from build123d import *

# Parameters (mm, degrees)
SKETCH_1_W                  = 30
SKETCH_1_H                  = 57
EXTRUDE_1_DEPTH             = 25
SKETCH_2_W                  = 5
SKETCH_2_H                  = 52
CUT_EXTRUDE_1_DEPTH         = 65.02343321
SKETCH_3_W                  = 5
SKETCH_3_H                  = 52
CUT_EXTRUDE_2_DEPTH         = 65.02343321
SKETCH_4_W                  = 20
SKETCH_4_H                  = 38
EXTRUDE_2_DEPTH             = 20
SKETCH_5_W                  = 28.836169251
SKETCH_5_H                  = 18
CUT_EXTRUDE_3_DEPTH         = 69.190018281
HOLE_WIZARD_10_0_10_1_D     = 10
HOLE_WIZARD_10_0_10_1_DEPTH = 10
HOLE_WIZARD_10_0_10_2_D     = 10
HOLE_WIZARD_10_0_10_2_DEPTH = 38
HOLE_WIZARD_5_0_5_1_D       = 5
HOLE_WIZARD_5_0_5_1_DEPTH   = 17
HOLE_WIZARD_5_0_5_1_TIP     = 1.502151548
CHAMFER_1_SIZE              = 1
CHAMFER_2_SIZE              = 10
FILLET_1_R                  = 5


with BuildPart() as part:
    # 草图1 → 凸台-拉伸1 (new body)
    with BuildSketch(Plane(origin=(17.145402657, 0, 0), x_dir=(0, 0, -1), z_dir=(1, 0, 0))):
        with Locations((0, 28.5)):
            Rectangle(SKETCH_1_W, SKETCH_1_H)
    extrude(amount=-EXTRUDE_1_DEPTH)

    # 草图2 → 切除-拉伸1 (cut, through all)
    with BuildSketch(Plane(origin=(17.145402657, 0, 0), x_dir=(0, 0, -1), z_dir=(1, 0, 0))):
        with Locations((-12.5, 31)):
            Rectangle(SKETCH_2_W, SKETCH_2_H)
    extrude(amount=-CUT_EXTRUDE_1_DEPTH, mode=Mode.SUBTRACT)

    # 草图3 → 切除-拉伸2 (cut, through all)
    with BuildSketch(Plane(origin=(17.145402657, 0, 0), x_dir=(0, 0, -1), z_dir=(1, 0, 0))):
        with Locations((12.5, 31)):
            Rectangle(SKETCH_3_W, SKETCH_3_H)
    extrude(amount=-CUT_EXTRUDE_2_DEPTH, mode=Mode.SUBTRACT)

    # 草图4 → 凸台-拉伸2 (add)
    with BuildSketch(Plane.ZY.offset(7.854597343)):
        with Locations((0, 38)):
            Rectangle(SKETCH_4_W, SKETCH_4_H)
    extrude(amount=EXTRUDE_2_DEPTH)

    # 草图5 → 切除-拉伸3 (cut, through all)
    with BuildSketch(Plane.XY.offset(10)):
        with Locations((-13.436512718, 38)):
            Rectangle(SKETCH_5_W, SKETCH_5_H)
    extrude(amount=-CUT_EXTRUDE_3_DEPTH, mode=Mode.SUBTRACT)

    # Ø10.0 (10) 直径孔1
    with Locations(Plane(origin=(0, 47, 0), x_dir=(-1, 0, 0), z_dir=(0, -1, 0))):
        with Locations((17.854597343, 0)):
            Hole(HOLE_WIZARD_10_0_10_1_D / 2, depth=HOLE_WIZARD_10_0_10_1_DEPTH)

    # Ø10.0 (10) 直径孔2
    with Locations(Plane(origin=(0, 19, 0), x_dir=(-1, 0, 0), z_dir=(0, -1, 0))):
        with Locations((17.854597343, 0)):
            Hole(HOLE_WIZARD_10_0_10_2_D / 2, depth=HOLE_WIZARD_10_0_10_2_DEPTH)

    # Ø5.0 (5) 直径孔1
    with Locations(Plane(origin=(0, 0, 0), x_dir=(-1, 0, 0), z_dir=(0, -1, 0))):
        with Locations((2.854597343, 0), (-12.145402657, 0)):
            Hole(HOLE_WIZARD_5_0_5_1_D / 2, depth=HOLE_WIZARD_5_0_5_1_DEPTH)
            with Locations((0, 0, -(HOLE_WIZARD_5_0_5_1_DEPTH + HOLE_WIZARD_5_0_5_1_TIP / 2))):  # 118° drill point
                Cone(0, HOLE_WIZARD_5_0_5_1_D / 2, HOLE_WIZARD_5_0_5_1_TIP, mode=Mode.SUBTRACT)

    # 倒角1
    chamfer_1_edges = [part.edges().sort_by_distance(p)[0] for p in [
        (-27.854597343, 52, -10),
        (-27.854597343, 24, 10),
        (-27.854597343, 24, -10),
        (-27.854597343, 52, 10),
    ]]
    chamfer(chamfer_1_edges, length=CHAMFER_1_SIZE)

    # 倒角2
    chamfer_2_edges = [part.edges().sort_by_distance(p)[0] for p in [
        (17.145402657, 57, 0),
    ]]
    chamfer(chamfer_2_edges, length=CHAMFER_2_SIZE)

    # 圆角1
    fillet_1_edges = [part.edges().sort_by_distance(p)[0] for p in [
        (0.981571908, 47, 0),
        (0.981571908, 29, 0),
    ]]
    fillet(fillet_1_edges, radius=FILLET_1_R)


solid = part.part
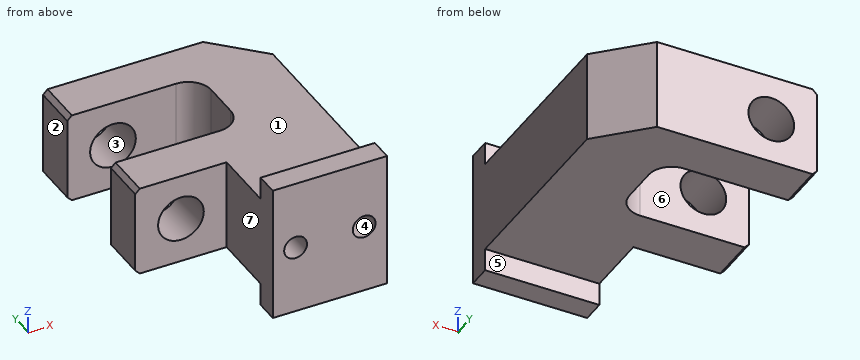
For this review, take the finished solid that the model builds, in its own axes (mm). Face numbers are marked on the shaded views. A direction names the side the tool comes from. Round coordinates to 2 decimals unless told otherwise and drop trailing zeros. Order: outer loops, then holes, each group sorted by start corner. A loop starts at its lowest first (then second) coordinate and runs counter-clockwise, first axis right, second up. Notation, with made-up numbers: M 26,78 L 44,78 A32 ccw 44,106 Z; hole C 69.25,6 d3. An arc over 180 degrees is marked long. Write each question's results on one line, items separated by ' | '. Start each with the question number.
1. Add section D-D (x = -18). State the section outline as (y, z) points, then the cut area to 3 significant figures.
2. Add section A-A (x = -23.5). State the section outline as (y, z) points.
3. Draft analysis for pull direction X (two halves, no side actions). For the marked faces 1, 2 and 3, state which applies: pulls with the +X half, pulls with the -X half, needs draft (parallel to the pull), parting line crosses it, or undercut.
4. To check wall thickness, follow L1, parallel to Y at x = -24.5, z = 9; L2, parallel to X at y = 39, z = 4.5; L3, parallel to X at y = 48, z = -0.5. State the ranges of each line that lie inside material, in increasing order. Write a range as [from, to].
5. Add section B-B (y = 13). State the section outline as (x, z) points, then the cut area to 3 significant figures.
6. Tool access review of the marked faces 4, 5, 6 and 7: name each direction out of +Z, -Z, +X, -X, +Y, -Y from which nothing blocks a thin tool from reaching the whole face with its end or side.
7. Clearance check with flat-ended pins moving along their axes: pin 1 Ø6 at (x, z) = (-17.85, 0) entering from -Y; pin 2 Ø6.5 at (y, z) = (38, -3) entering from -X; pin 3 Ø10 at (x, z) = (-18, -2.5) entering from -Y; pin 4 Ø22 at (x, y) = (-1, 39.5) entering from -Z. State where each tip first meets the part, or that it passes through.
8. Add section C-C (z = 5.75). State the section outline as (x, y) points, then the cut area to 3 significant figures.
Output values:
1) outline: M 19,-10 L 29,-10 L 29,-5 L 19,-5 Z; M 19,5 L 29,5 L 29,10 L 19,10 Z; M 47,-10 L 57,-10 L 57,-5 L 47,-5 Z; M 47,5 L 57,5 L 57,10 L 47,10 Z | area: 200 mm^2
2) outline: M 19,-10 L 29,-10 L 29,10 L 19,10 Z; M 47,-10 L 57,-10 L 57,10 L 47,10 Z
3) face 1: needs draft | face 2: pulls with the -X half | face 3: undercut
4) L1: [19, 29], [47, 57] | L2: [0.98, 17.15] | L3: [-27.85, -22.83], [-12.88, 16.15]
5) outline: M -7.85,-10 L 17.15,-10 L 17.15,10 L -7.85,10 Z; hole C -2.85,0 d5; hole C 12.15,0 d5 | area: 461 mm^2
6) face 4: -Y | face 5: -Z, +X, -X, +Y | face 6: +Z, -Z, -X | face 7: +Z, -Z, -X, -Y
7) pin 1: through | pin 2: x = 0.98 | pin 3: y = 19 | pin 4: z = -10
8) outline: M -27.85,19 L -7.85,19 L -7.85,0 L 17.15,0 L 17.15,47 L 7.15,57 L -27.85,57 L -27.85,47 L -4.02,47 A5 cw 0.98,42 L 0.98,34 A5 cw -4.02,29 L -27.85,29 Z | area: 1,630 mm^2
